from build123d import *

# Parameters (mm, degrees)
EDGE_CHAMFER_0_0625IN_X_45DEG_SIZE = 1.5875


with BuildPart() as part:
    # Bushing Profile Sketch → Flanged Bushing Revolve (revolve)
    with BuildSketch(Plane.XY, mode=Mode.PRIVATE) as flanged_bushing_revolve_sk:
        Polygon((15.875, 6.35), (-15.875, 6.35), (-15.875, 8.89), (-15.875, 9.525), (-14.2875, 9.525), (-12.7, 9.525), (-12.7, 7.75), (15.875, 7.75), align=None)
    revolve(flanged_bushing_revolve_sk.sketch.rotate(Axis((40.781111111, 0, 0), (-1, 0, 0)), 90), axis=Axis((40.781111111, 0, 0), (-1, 0, 0)))

    # Edge Chamfer 0.0625in x 45deg
    edge_chamfer_0_0625in_x_45deg_edges = [part.edges().sort_by_distance(p)[0] for p in [
        (-15.875, 0, 9.525),
    ]]
    chamfer(edge_chamfer_0_0625in_x_45deg_edges, length=EDGE_CHAMFER_0_0625IN_X_45DEG_SIZE)


solid = part.part
Design review of the part built by this model. Coordinates are the model's own, in mm. A direction names the side the tool comes from. Give positions to 0.01 mm unless a question says otherwise; leave off trailing zeros. Order: outer loops, then holes, each group sorted by start corner. A loop starts at its lowest first (then second) coordinate and runs counter-clockwise, first axis right, second up.
1. Tool access review of faces 1 (the flat face through (-12.7, 8, -1)), 2 (the cylindrical face through (-13.5, 9.3, 2.06)): name each direction out of +Z, -Z, +X, -X, +Y, -Y from which nothing blocks a thin tool from reaching the whole face with its end or side.
Solution:
face 1: +X
face 2: +X, -X
2. To check wall thickness, follow L1, parallel to Y at x = 2, z = 0; L2, parallel to Y at x = -9.5, z = 5.75; L3, parallel to Z at x = -13, y = 1.25. State the ranges of each line that lie inside material, in increasing order.
Solution:
L1: y = -7.75 to -6.35, 6.35 to 7.75
L2: y = -5.2 to -2.69, 2.69 to 5.2
L3: z = -9.44 to -6.23, 6.23 to 9.44
3. Mouldability with a two-part tool opening along Z and no side actions: class faces 3 (the flat face through (-15.875, -7, 0)), 4 (the cylindrical face through (-0.22, 3.86, 5.04)), 5 (the cylindrical face through (1.788, -7.684, 1.009)) as +Z half, -Z half, draft (parallel to the pull), parting line (faces both ways), or undercut.
Solution:
face 3: draft
face 4: undercut
face 5: parting line
4. Add section C-C, the plane x = -5. State the section outline as (y, z) points.
Solution:
outline: circle Ø15.5 at (0, 0); hole circle Ø12.7 at (0, 0)
5. For pin 1 Ø10 at (x, z) = (10, -5.5) entering from -Y; pin 2 Ø10 at (x, y) = (4.5, -3) entering from -Z; pin 3 Ø8 at (x, z) = (5.5, -4) entering from +Y, all flat-tipped, find the tip position at first contact; note any pin that passes through.
Solution:
pin 1: stops at y = -7.73
pin 2: stops at z = -7.75
pin 3: stops at y = 7.75
